Build history of the part. All positions in model axes, mm. A direction names the side the tool comes from. Give positions to 0.01 mm unless a question says otherwise; leave off trailing zeros. Loops run counter-clockwise (first coordinate to the right, second up) from the corner with the lowest first, then second, coordinate; pieces in that order, holes last. Notation, with made-up numbers: (82.5, 59) - (102.5, 59) arc R35 cw to (102.5, 95) - close; hole circle Ø2 at (15.25, 1.25). An arc over 180 degrees is marked (long way). Return JSON: item names as keys, results as strings. Group by question number.
1) Slice it at C-C (x = -168.5). List the corners of the cut face in (y, z).
2) 3-axis set-ups, long thin cutter, end or side, ignore diameter. For faces 5 (the face through (550, 92, 26)), 6 (the face through (-427, -28, 25)), 7 (the face through (529, 372, 39)): which of +Z, -Z, +X, -X, +Y, -Y reach the whole face in a straight line?
3) Slice it at B-B (z = 34). List the corners of the cut face in (x, y) (3 decimals).
4) Drill centre lines: probe 1 along X at (y, z) = (199, 51.8); probe 2 along Y at (x, z) = (-316, 52); probe 3 along X at (y, z) = (20.5, 24). Where is each one in solid material? Low to high. Write a range as from..to.
5) Slice it at D-D (y = -337.5). List the corners of the cut face in (x, z).
6) Mould opens along Z. For faces 1 (the face through (517, 72, 29)), 2 (the face through (426.75, -287.74, 26.13)), 3 (the face through (529.303, -210.205, 38.783)), 4 (the face through (518.883, 72.836, 30.03)) say: released by +Z, released by -Z, zero draft, split by the parting line, or undercut.
7) Slice it at A-A (y = 111.5). List the corners of the cut face in (x, z).
8) Drop flat-ended pins along their axis: pin 1 (8 mm diameter, centred on x = 155, z = 41.5, fed in from -Y); pin 2 (12 mm diameter, centred on x = 199, y = 103, fed in from -Z); pin 3 (1 mm diameter, centred on x = 382.5, z = 27, fed in from -Y). Give the stop position or say it passes through.
```python
from build123d import *

# Parameters (mm, degrees)
EXTRUDE_1_DEPTH        = 53
EXTRUDE_1_2_DEPTH      = 3
EXTRUDE_2_DEPTH        = 50
EXTRUDE_3_REACH        = 966.878
CUT_EXTRUDE_1_REACH    = 695.448
SKETCH_5_R             = 4.1
HOLE_WIZARD_M8_1_D     = 6.8
HOLE_WIZARD_M8_1_DEPTH = 8
HOLE_WIZARD_M5_1_D     = 4.2
HOLE_WIZARD_M5_1_DEPTH = 14
HOLE_WIZARD_M5_1_TIP   = 1.2618073


with BuildPart() as part:
    # 草图1 → Extrude 1 (new body)
    with BuildSketch(Plane.XY):
        Polygon((-430, 375), (-111, 375), (550, 375), (550, -199), (300, -379), (-100, -419), (-430, -419), align=None)
        Polygon((-427, 372), (-111, 372), (547, 372), (547, -197.463298768), (298.9004217, -376.094995144), (-100.149626863, -416), (-427, -416), align=None, mode=Mode.SUBTRACT)
    extrude(amount=EXTRUDE_1_DEPTH)

    # 草图2 → Extrude 1 2 (add)
    with BuildSketch(Plane(origin=(0, 0, 53), x_dir=(-1, 0, 0), z_dir=(0, 0, -1))):
        Polygon((100, -419), (430, -419), (430, 375), (-550, 375), (-550, -199), (-300, -379), align=None)
    extrude(amount=EXTRUDE_1_2_DEPTH)

    # 草图3 → 凸台-拉伸2 (add)
    with BuildSketch(Plane(origin=(0, 0, 50), x_dir=(-1, 0, 0), z_dir=(0, 0, -1))):
        Polygon((-542, 375), (-550, 375), (-550, -199), (-544.865692733, -199), (-542, -201.063298768), (-542, -199.063298768), align=None)
    extrude(amount=EXTRUDE_2_DEPTH)

    # 拉伸-薄壁3: up to this plane
    extrude_3_end = Plane(origin=(280.386179605, -389.425249452, 53), z_dir=(-0.584304725845076, 0.8115343414514945, 0))
    # 草图4 → 拉伸-薄壁3 (add, up to the surface)
    with BuildSketch(Plane.XZ.offset(-372), mode=Mode.PRIVATE) as extrude_3_sk1:
        Polygon((492, 50), (542, 8), (543.286384173, 9.53140973), (493.286384173, 51.53140973), align=None)
    extrude_3_tool1 = split(extrude(extrude_3_sk1.sketch, amount=EXTRUDE_3_REACH, mode=Mode.PRIVATE), bisect_by=extrude_3_end, keep=Keep.BOTH, mode=Mode.PRIVATE)
    add(extrude_3_tool1.solids().sort_by_distance((517.643192, 372, 29.765705))[0])

    # 草图5 → 切除-拉伸1 (cut, up to next)
    with BuildSketch(Plane.XY.offset(53), mode=Mode.PRIVATE) as cut_extrude_1_sk1:
        with Locations((-316.5, 82.25)):
            Circle(SKETCH_5_R)
    cut_extrude_1_tool1 = extrude(cut_extrude_1_sk1.sketch, amount=-CUT_EXTRUDE_1_REACH, mode=Mode.PRIVATE) & part.part
    # 草图5 → 切除-拉伸1 (cut, up to next)
    with BuildSketch(Plane.XY.offset(53), mode=Mode.PRIVATE) as cut_extrude_1_sk2:
        with Locations((-316.5, -34.25)):
            Circle(SKETCH_5_R)
    cut_extrude_1_tool2 = extrude(cut_extrude_1_sk2.sketch, amount=-CUT_EXTRUDE_1_REACH, mode=Mode.PRIVATE) & part.part
    add(cut_extrude_1_tool1.solids().sort_by_distance((-316.5, 82.25, 53))[0], mode=Mode.SUBTRACT)
    add(cut_extrude_1_tool2.solids().sort_by_distance((-316.5, -34.25, 53))[0], mode=Mode.SUBTRACT)

    # M8 螺纹孔1
    with Locations(Plane(origin=(550, 0, 0), x_dir=(0, 0, -1), z_dir=(1, 0, 0))):
        with Locations((-21, 315), (-21, 285), (-21, 45), (-21, 15)):
            Hole(HOLE_WIZARD_M8_1_D / 2, depth=HOLE_WIZARD_M8_1_DEPTH)

    # M5 螺纹孔1
    with Locations(Plane.XY.offset(53)):
        with Locations((-415.514659804, 199), (-382.014659804, 199), (-415.514659804, -81), (-382.014659804, -81)):
            Hole(HOLE_WIZARD_M5_1_D / 2, depth=HOLE_WIZARD_M5_1_DEPTH)
            with Locations((0, 0, -(HOLE_WIZARD_M5_1_DEPTH + HOLE_WIZARD_M5_1_TIP / 2))):  # 118° drill point
                Cone(0, HOLE_WIZARD_M5_1_D / 2, HOLE_WIZARD_M5_1_TIP, mode=Mode.SUBTRACT)


solid = part.part
```
Results:
{
 "1": {"outline": "(-419, 0) - (-416, 0) - (-416, 50) - (372, 50) - (372, 0) - (375, 0) - (375, 53) - (-419, 53) - close"},
 "2": {"face 5": "+Z, -Z, +X, +Y, -Y", "face 6": "-Z", "face 7": "none"},
 "3": {"outline": "(-430, -419) - (-100, -419) - (300, -379) - (550, -199) - (550, 375) - (-430, 375) - close; hole (-427, -416) - (-100.15, -416) - (298.9, -376.095) - (511.048, -223.349) - (511.048, 372) - (-427, 372) - close; hole (514.157, -221.11) - (542, -201.063) - (542, 372) - (514.157, 372) - close"},
 "4": {"probe 1": "-430..-417.61, -413.41..-384.11, -379.91..550", "probe 2": "-419..-38.32, -30.18..78.18, 86.32..375", "probe 3": "-430..-427, 522.95..526.06, 542..550"},
 "5": {"outline": "(-430, 0) - (-427, 0) - (-427, 50) - (352.5, 50) - (352.5, 0) - (357.64, 0) - (357.64, 53) - (-430, 53) - close"},
 "6": {"face 1": "released by -Z", "face 2": "zero draft", "face 3": "undercut", "face 4": "undercut"},
 "7": {"outline": "(-430, 0) - (-427, 0) - (-427, 50) - (492, 50) - (542, 8) - (542, 0) - (550, 0) - (550, 53) - (-430, 53) - close; hole (495.11, 50) - (542, 10.61) - (542, 50) - close"},
 "8": {"pin 1": "y = -393.9", "pin 2": "z = 50", "pin 3": "y = -319.96"}
}
